Geometry check sheet. Reference: the model listing, model coordinates, mm. Give positions to 0.01 mm unless a question says otherwise; leave off trailing zeros. Write each loop counter-clockwise with the first axis right and the second up, starting at its lowest first coordinate (ties: lowest second). Pieces come first, ordered by that corner, then holes. Notation, with made-up numbers: (7, 38.25) -> (66, 38.25) arc R14 cw to (66, 51.25) -> close; hole circle Ø9 at (42.25, -0.5). An arc over 180 degrees is marked (long way). Write item = value, one per line. Start each with the question number.
1. Cross-section at B-B, the plane y = 0. Record the cut outline in (x, z), plus the area to 3 significant figures.
2. Cross-section at A-A, the plane z = -58. Record the cut outline in (x, y), plus the area to 3 significant figures.
3. Thickness scan on line 1 along Y through (x, z) = (-5, -58); line 2 along Y through (x, z) = (5, -21.5). Record the ranges inside material, lowest first.
4. Mould release check, pull along Z, two halves, no side actions. Record for faces 1 (the cylindrical face through (-0.21, -4.868, -64.349)), 2 (the flat face through (0, 0, -83)), 3 (the flat face through (0, -30, 285)), 4 (the flat face through (0, 0, 642)): pulls with the +Z half, pulls with the -Z half, needs draft (parallel to the pull), parting line crosses it, or undercut.
```python
from build123d import *

# Parameters (mm, degrees)
SKETCH_1_W          = 30
SKETCH_1_H          = 60
EXTRUDE_1_DEPTH     = 642
SKETCH_2_W          = 30
SKETCH_2_H          = 60
EXTRUDE_2_DEPTH     = 83
SKETCH_3_R          = 8
CUT_EXTRUDE_1_DEPTH = 644.400341933


with BuildPart() as part:
    # 草图1 → 凸台-拉伸1 (new body)
    with BuildSketch(Plane.XY):
        Rectangle(SKETCH_1_W, SKETCH_1_H)
    extrude(amount=EXTRUDE_1_DEPTH)

    # 草图2 → 凸台-拉伸2 (add)
    with BuildSketch(Plane(origin=(0, 0, 0), x_dir=(-1, 0, 0), z_dir=(0, 0, -1))):
        Rectangle(SKETCH_2_W, SKETCH_2_H)
    extrude(amount=EXTRUDE_2_DEPTH)

    # 草图3 → 切除-拉伸1 (cut, through all)
    with BuildSketch(Plane.ZY.offset(15)):
        with Locations((-58, 0)):
            Circle(SKETCH_3_R)
        with Locations((-23, 0)):
            Circle(SKETCH_3_R)
    extrude(amount=-CUT_EXTRUDE_1_DEPTH, mode=Mode.SUBTRACT)


solid = part.part
```
Answers:
q1.outline = (-15, -83) -> (15, -83) -> (15, -66) -> (-15, -66) -> close; (-15, -50) -> (15, -50) -> (15, -31) -> (-15, -31) -> close; (-15, -15) -> (15, -15) -> (15, 642) -> (-15, 642) -> close
q1.area = 20,800 mm^2
q2.outline = (-15, -30) -> (15, -30) -> (15, -8) -> (-15, -8) -> close; (-15, 8) -> (15, 8) -> (15, 30) -> (-15, 30) -> close
q2.area = 1,320 mm^2
q3.line_1 = -30 to -8, 8 to 30
q3.line_2 = -30 to -7.86, 7.86 to 30
q4.face_1 = undercut
q4.face_2 = pulls with the -Z half
q4.face_3 = needs draft
q4.face_4 = pulls with the +Z half
